For this review, use the dimensioned drawing (mm, ordinates from the lowest corner) and the shaded views. A direction names the side the tool comes from. Coordinates: 2 decimals unless noted, no trailing zeros. Loops run counter-clockwise (first coordinate to the right, second up) from the corner with the lowest first, then second, coordinate; pieces in that order, holes last. Notation, with made-up numbers: M 7.5,31 L 64.5,31 A23 ccw 64.5,50 Z; hole C -20,66.25 d11. An arc over 180 degrees is marked long. One line per item, written item: value.
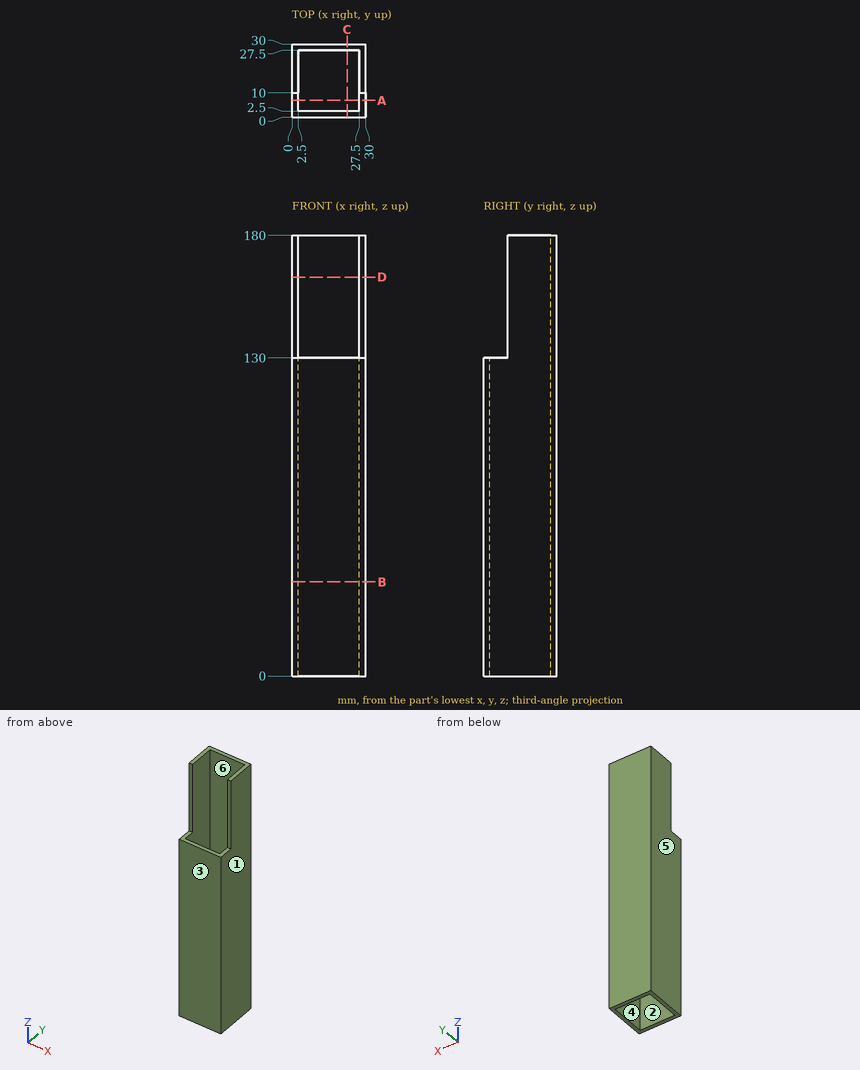
(1) Insertion check: pin 1 (8 mm diameter, centred on x = 16, y = 3.5, fed in from +Z); pin 2 (2 mm diameter, centred on x = 1.5, z = 157, fed in from -Y). Each pin has a flat end and moves straight along its axis. Give the tip position at first contact, or say it passes through.
Reply:
pin 1: stops at z = 130
pin 2: stops at y = 10
(2) Mouldability with a two-part tool opening along X and no side actions: class the marked faces 1, 2, 3 and 4 as released by +X, released by -X, zero draft, split by the parting line, or undercut.
Reply:
face 1: released by +X
face 2: undercut
face 3: zero draft
face 4: undercut
(3) We need section C-C on x = 22.5. State the section outline as (y, z) points.
Reply:
outline: M 0,0 L 2.5,0 L 2.5,130 L 0,130 Z; M 27.5,0 L 30,0 L 30,180 L 27.5,180 Z
(4) We need section D-D on z = 163. State the section outline as (x, y) points, then the cut area to 4 significant figures.
Reply:
outline: M 0,10 L 2.5,10 L 2.5,27.5 L 27.5,27.5 L 27.5,10 L 30,10 L 30,30 L 0,30 Z
area: 162.5 mm2
(5) We need section A-A on y = 7. State the section outline as (x, z) points, then the cut area to 3 significant figures.
Reply:
outline: M 0,0 L 2.5,0 L 2.5,130 L 0,130 Z; M 27.5,0 L 30,0 L 30,130 L 27.5,130 Z
area: 650 mm2
(6) To check wall thickness, follow line 1 along Y through (x, z) = (15, 14.5); line 2 along Y through (x, z) = (24, 148). State the ranges of each line that lie inside material, in increasing order. Write a range as [from, to].
Reply:
line 1: y = [0, 2.5], [27.5, 30]
line 2: y = [27.5, 30]
(7) We need section B-B on z = 38.5. State the section outline as (x, y) points, then the cut area to 3 significant figures.
Reply:
outline: M 0,0 L 30,0 L 30,30 L 0,30 Z; hole M 2.5,2.5 L 27.5,2.5 L 27.5,27.5 L 2.5,27.5 Z
area: 275 mm2
(8) Tool access review of the marked faces 5 and 6: name each direction out of +Z, -Z, +X, -X, +Y, -Y from which nothing blocks a thin tool from reaching the whole face with its end or side.
Reply:
face 5: +Z, -Z, -X, +Y, -Y
face 6: +Z, -Z
